Design review of the part built by this model. Coordinates are the model's own, in mm. A direction names the side the tool comes from. Give positions to 0.01 mm unless a question says otherwise; leave off trailing zeros. Write each loop counter-clockwise with the first axis right and the second up, starting at its lowest first coordinate (ties: lowest second). Pieces come first, ordered by that corner, then holes.
```python
from build123d import *

# Parameters (mm, degrees)
BOSS_EXTRUDE1_DEPTH                     = 24
BOSS_EXTRUDE1_DEPTH_BACK                = 2
SKETCH1_W                               = 37.5
SKETCH1_H                               = 104.65705171
SKETCH2_W                               = 35
SKETCH2_H                               = 2
CUT_EXTRUDE1_DEPTH                      = 110.129961388
CHAMFER1_SIZE                           = 10
CBORE_FOR_M3_HEX_HEAD_BOLT1_D           = 3.4
CBORE_FOR_M3_HEX_HEAD_BOLT1_CBORE_D     = 9
CBORE_FOR_M3_HEX_HEAD_BOLT1_CBORE_DEPTH = 0.5


with BuildPart() as part:
    # Sketch1 → Boss-Extrude1 (new, two sides: drawn at the far end of the back side and taken through both)
    with BuildSketch(Plane.XY.offset(-BOSS_EXTRUDE1_DEPTH_BACK)):
        with Locations((-0.75, -2.428525855)):
            Rectangle(SKETCH1_W, SKETCH1_H)
    extrude(amount=BOSS_EXTRUDE1_DEPTH + BOSS_EXTRUDE1_DEPTH_BACK)

    # Sketch2 → Cut-Extrude1 (cut, through all)
    with BuildSketch(Plane.XZ.offset(54.75705171)):
        with Locations((0.5, -1)):
            Rectangle(SKETCH2_W, SKETCH2_H)
    extrude(amount=-CUT_EXTRUDE1_DEPTH, mode=Mode.SUBTRACT)

    # Chamfer1
    chamfer1_edges = [part.edges().sort_by_distance(p)[0] for p in [
        (18, -54.75705171, 12),
        (-19.5, -54.75705171, 11),
        (18, 49.9, 12),
        (-19.5, 49.9, 11),
    ]]
    chamfer(chamfer1_edges, length=CHAMFER1_SIZE)

    # CBORE for M3 Hex Head Bolt1 (through all)
    with Locations(Plane.XY.offset(24)):
        with Locations((-13, 32.7), (13, 32.7), (13, 6.7), (-13, 6.7), (-13, -11.55705171), (13, -11.55705171), (13, -37.55705171), (-13, -37.55705171)):
            CounterBoreHole(CBORE_FOR_M3_HEX_HEAD_BOLT1_D / 2, CBORE_FOR_M3_HEX_HEAD_BOLT1_CBORE_D / 2, CBORE_FOR_M3_HEX_HEAD_BOLT1_CBORE_DEPTH)


solid = part.part
```
(1) Tool access review of faces 4 (the face through (0, -3, 0)), 5 (the face through (18, -3, 12)), 6 (the face through (-10.581, 36.494, 23.754)): name each direction out of +Z, -Z, +X, -X, +Y, -Y from which nothing blocks a thin tool from reaching the whole face with its end or side.
Resolved:
face 4: -Z, +X, +Y, -Y
face 5: +Z, -Z, +X, +Y, -Y
face 6: +Z
(2) Consider section B-B, the plane z = 20. Give the number of separate pieces and of enclosed holes in the cut face, then the cut area to 3 significant figures.
Resolved:
separate pieces: 1
enclosed holes: 8
area: 3,650 mm2
(3) Consider section C-C, the plane x = -7. Give the boundary of the cut face in (y, z), then the cut area to 3 significant figures.
Resolved:
outline: (-54.76, 0) - (49.9, 0) - (49.9, 24) - (-54.76, 24) - close
area: 2,510 mm2
(4) Clearance check with flat-ended pins moving along their axes: P1, Ø4, axis at x = 13, y = -37.56, coming from the -Z side; P2, Ø7, axis at x = 13, y = -11.56, coming from the +Z side. State where each tip first meets the part, or that it passes through.
Resolved:
P1: stops at z = 0
P2: stops at z = 23.5
(5) Consider section A-A, the plane y = 32.7. Give the boundary of the cut face in (x, z).
Resolved:
outline: (-19.5, -2) - (-17, -2) - (-17, 0) - (-14.7, 0) - (-14.7, 23.5) - (-17.5, 23.5) - (-17.5, 24) - (-19.5, 24) - close; (-11.3, 0) - (11.3, 0) - (11.3, 23.5) - (8.5, 23.5) - (8.5, 24) - (-8.5, 24) - (-8.5, 23.5) - (-11.3, 23.5) - close; (14.7, 0) - (18, 0) - (18, 24) - (17.5, 24) - (17.5, 23.5) - (14.7, 23.5) - close
(6) To check wall thickness, follow L1, parallel to Y at x = -13, z = 19; L2, parallel to Y at x = 13, z = 8.25; L3, parallel to Z at x = -1, y = -5. State the ranges of each line that lie inside material, in increasing order.
Resolved:
L1: y = -51.26 to -39.26, -35.86 to -13.26, -9.86 to 5, 8.4 to 31, 34.4 to 46.4
L2: y = -49.76 to -39.26, -35.86 to -13.26, -9.86 to 5, 8.4 to 31, 34.4 to 44.9
L3: z = 0 to 24
(7) Mouldability with a two-part tool opening along X and no side actions: class faces 1 (the face through (12.086, 34.133, 11.586)), 2 (the face through (-18, -2, -2)), 3 (the face through (13.1, 44.8, 11.8)) as pulls with the +X half, pulls with the -X half, needs draft (parallel to the pull), parting line crosses it, or undercut.
Resolved:
face 1: undercut
face 2: needs draft
face 3: pulls with the +X half
